Geometry check sheet. Reference: the model listing, model coordinates, mm. Face numbers are marked on the shaded views. Round coordinates to 2 decimals unless told otherwise and drop trailing zeros. Loops run counter-clockwise (first coordinate to the right, second up) from the corner with the lowest first, then second, coordinate; pieces in that order, holes last. Notation, with made-up numbers: (5, 87.25) -> (25, 87.25) arc R15 cw to (25, 116.25) -> close; hole circle Ø3 at (-30, 54). An arc over 180 degrees is marked (long way). Use a Markdown table: item, result. Add a question column.
Q1. Material ranges on L1, parallel to X at y = 0.7, z = 0; L2, parallel to X at y = -2.5, z = 0; L3, parallel to X at y = 1.5, z = 0, recorded low to high.
Q2. Release check for a two-part mould opening along X. For the marked faces 1, 2 and 3 record: released by +X, released by -X, zero draft, split by the parting line, or undercut.
Q3. Sectioned sample at A-A, the plane z = 0. Enter the section's corners in (x, y), then the cut area to 3 significant figures.
Q4. Sectioned sample at C-C, the plane y = 3.5. Enter the section's corners in (x, z).
Q5. Gauge pin test, flat ends, axial feed: P1, Ø6, axis at y = -4, z = 15.5, coming from the +X side; P2, Ø3, axis at x = 22, y = -3.5, coming from the -Z side; P3, Ø1, axis at x = 9, y = -2.5, coming from the -Z side. Record the tip position at first contact, or that the pin passes through.
Q6. Sectioned sample at B-B, the plane x = 0. Enter the section's corners in (y, z).
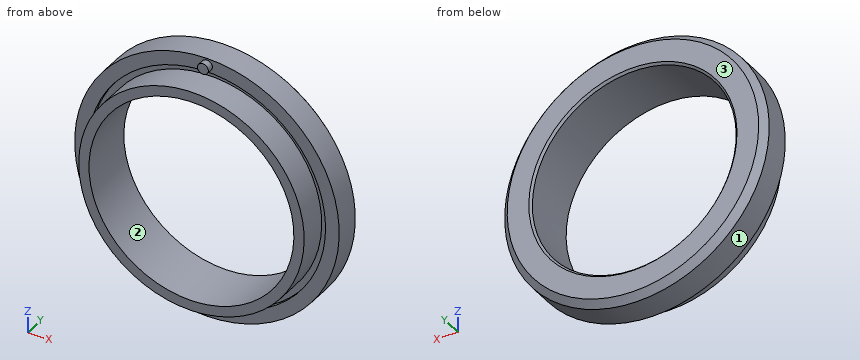
```python
from build123d import *

# Parameters (mm, degrees)
CUT_EXTRUDE_1_DEPTH      = 44.780703512
CUT_EXTRUDE_1_DEPTH_BACK = 44.780703512
CHAMFER_1_SIZE           = 0.5
CHAMFER_2_SIZE           = 1.5
SKETCH_3_R               = 1.25
EXTRUDE_1_DEPTH          = 1.5


with BuildPart() as part:
    # 草图1 → 旋转1 (revolve)
    with BuildSketch(Plane.XY, mode=Mode.PRIVATE) as revolve_1_sk:
        Polygon((23.5, -7.5), (23.5, 7.5), (30.5, 7.5), (30.5, 0), (27.35, 0), (27.35, 1), (25.85, 1), (25.85, -7.5), align=None)
    revolve(revolve_1_sk.sketch.rotate(Axis((0, 0, 0), (0, 1, 0)), 90), axis=Axis((0, 0, 0), (0, 1, 0)))

    # 草图2 → 切除-拉伸1 (cut, two sides: drawn at the far end of the back side and taken through both)
    with BuildSketch(Plane.XY.offset(-CUT_EXTRUDE_1_DEPTH_BACK)):
        Polygon((-25.85, -6), (25.85, -5.548820935), (25.85, -7.5), (-25.85, -7.5), align=None)
    extrude(amount=CUT_EXTRUDE_1_DEPTH + CUT_EXTRUDE_1_DEPTH_BACK, mode=Mode.SUBTRACT)

    # 倒角1
    chamfer_1_edges = [part.edges().sort_by_distance(p)[0] for p in [
        (0, 7.5, 23.5),
    ]]
    chamfer(chamfer_1_edges, length=CHAMFER_1_SIZE)

    # 倒角2
    chamfer_2_edges = [part.edges().sort_by_distance(p)[0] for p in [
        (0, 7.5, 30.5),
    ]]
    chamfer(chamfer_2_edges, length=CHAMFER_2_SIZE)

    # 草图3 → 凸台-拉伸1 (add)
    with BuildSketch(Plane.XZ):
        with Locations(Location((0, 28.85, 0), (0, 0, 270))):
            Circle(SKETCH_3_R)
    extrude(amount=EXTRUDE_1_DEPTH)


solid = part.part
```
Values:
| question | item | result |
|---|---|---|
| 1 | L1 | -30.5 to -27.35, -25.85 to -23.5, 23.5 to 25.85, 27.35 to 30.5 |
| 1 | L2 | -25.85 to -23.5, 23.5 to 25.85 |
| 1 | L3 | -30.5 to -23.5, 23.5 to 30.5 |
| 2 | face 1 | split by the parting line |
| 2 | face 2 | undercut |
| 2 | face 3 | zero draft |
| 3 | outline | (-30.5, 0) -> (-27.35, 0) -> (-27.35, 1) -> (-25.85, 1) -> (-25.85, -6) -> (-23.5, -5.98) -> (-23.5, 7) -> (-24, 7.5) -> (-29, 7.5) -> (-30.5, 6) -> close; (23.5, -5.57) -> (25.85, -5.55) -> (25.85, 1) -> (27.35, 1) -> (27.35, 0) -> (30.5, 0) -> (30.5, 6) -> (29, 7.5) -> (24, 7.5) -> (23.5, 7) -> close |
| 3 | area | 127 mm^2 |
| 4 | outline | circle Ø61 at (0, 0); hole circle Ø47 at (0, 0) |
| 5 | P1 | x = 22.63 |
| 5 | P2 | z = -15.75 |
| 5 | P3 | z = -24.41 |
| 6 | outline | (-5.77, -25.85) -> (1, -25.85) -> (1, -27.35) -> (0, -27.35) -> (0, -30.5) -> (6, -30.5) -> (7.5, -29) -> (7.5, -24) -> (7, -23.5) -> (-5.77, -23.5) -> close; (-5.77, 23.5) -> (7, 23.5) -> (7.5, 24) -> (7.5, 29) -> (6, 30.5) -> (0, 30.5) -> (0, 30.1) -> (-1.5, 30.1) -> (-1.5, 27.6) -> (0, 27.6) -> (0, 27.35) -> (1, 27.35) -> (1, 25.85) -> (-5.77, 25.85) -> close |
